Study the drawing (mm; zero at the part's minimum x, y, z) and answer. A direction names the side the tool comes from. Coordinates: 2 decimals unless noted, no trailing zeros. Order: outer loops, then holes, each group sorted by start corner. A loop starts at its lowest first (then second) coordinate and runs counter-clockwise, first axis right, second up. Notation, with made-up numbers: M -27,-24.75 L 27,-24.75 A22 ccw 27,-12.75 Z; hole C -7.75,-37.5 d3. An arc over 180 degrees is marked long. Put each result on its own line as item: value.
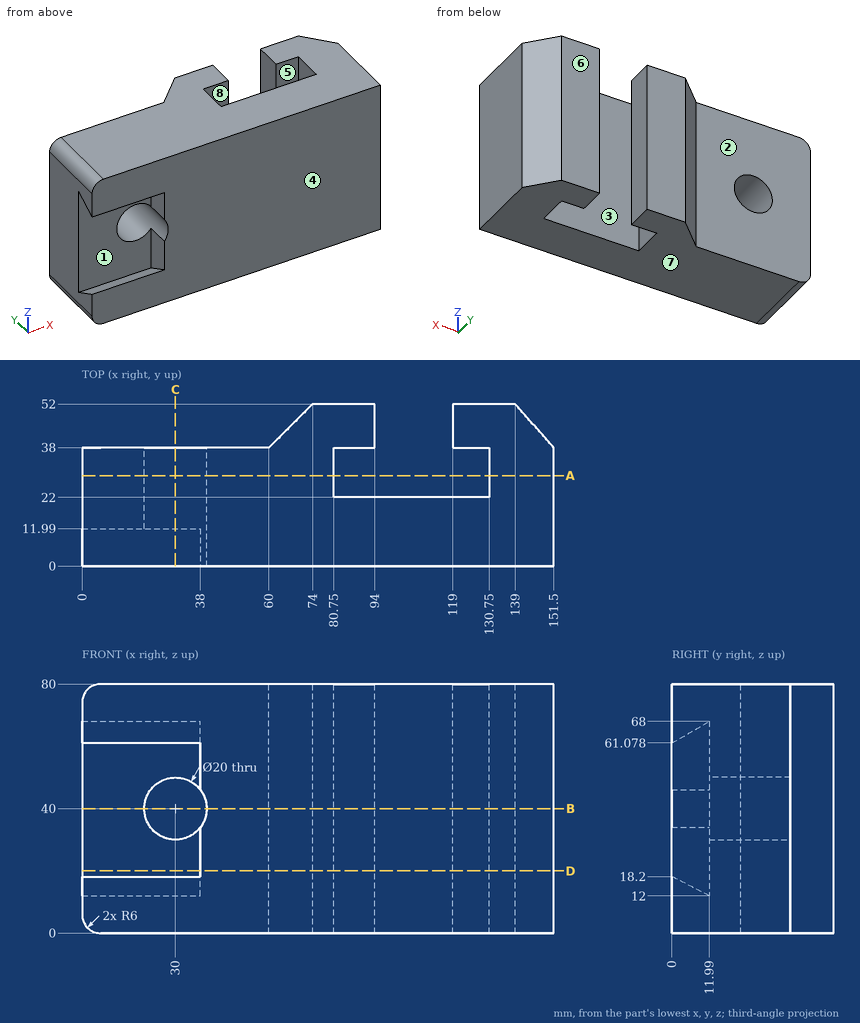
Q1. Consider line 1 along X through (y, z) = (29.5, 40); line 2 along X through (y, z) = (16, 40); line 3 along Y through (x, z) = (88.5, 76). Determine where each line is inside the solid, lowest interval first.
Answers below:
line 1: x = 0 to 20, 40 to 80.75, 130.75 to 151.5
line 2: x = 0 to 20, 40 to 151.5
line 3: y = 0 to 22, 38 to 52
Q2. Find section D-D on z = 20. Write down the section's boundary in (x, y), plus the area to 3 significant figures.
Answers below:
outline: M 0,11.99 L 38,11.99 L 38,0 L 151.5,0 L 151.5,38 L 139,52 L 119,52 L 119,38 L 130.75,38 L 130.75,22 L 80.75,22 L 80.75,38 L 94,38 L 94,52 L 74,52 L 60,38 L 0,38 Z
area: 5,250 mm^2
Q3. Find section B-B on z = 40. Write down the section's boundary in (x, y).
Answers below:
outline: M 0,11.99 L 20,11.99 L 20,38 L 0,38 Z; M 40,0 L 151.5,0 L 151.5,38 L 139,52 L 119,52 L 119,38 L 130.75,38 L 130.75,22 L 80.75,22 L 80.75,38 L 94,38 L 94,52 L 74,52 L 60,38 L 40,38 Z
Q4. Given pin 1 (11 mm diameter, centred on y = 48.5, z = 32.5, fed in from +X) (1 decimal); pin 2 (3.5 mm diameter, centred on y = 4.5, z = 18.5, fed in from -X); pin 3 (12 mm diameter, centred on x = 30, z = 40, fed in from +Y); pin 4 (19 mm diameter, centred on x = 20, z = 39, fed in from -Y), each flat-ended and moving along its own axis, determine where each tip first touches the part or whether it passes through.
Answers below:
pin 1: stops at x = 147
pin 2: stops at x = 38
pin 3: passes through
pin 4: stops at y = 11.99
Q5. Find section A-A on y = 29. Write down the section's boundary in (x, z).
Answers below:
outline: M 0,6 A6 ccw 6,0 L 80.75,0 L 80.75,80 L 6,80 A6 ccw 0,74 Z; M 130.75,0 L 151.5,0 L 151.5,80 L 130.75,80 Z; hole C 30,40 d20
Q6. Find section C-C on x = 30. Write down the section's boundary in (y, z), plus the area to 3 significant figures.
Answers below:
outline: M 0,0 L 38,0 L 38,30 L 11.99,30 L 11.99,12 L 0,18.2 Z; M 0,61.08 L 11.99,68 L 11.99,50 L 38,50 L 38,80 L 0,80 Z
area: 1,930 mm^2
Q7. A tool of negligible diameter and unlimited length cuts with its end or side. For the marked faces 1, 2, 3 and 4, from which of +Z, -Z, +X, -X, +Y, -Y can it reach the whole face along a straight path? Write none if from no direction.
Answers below:
face 1: -X
face 2: +Z, -Z, -X, +Y
face 3: +Z, -Z
face 4: +Z, -Z, +X, -X, -Y
Q8. For a pull along Y with two mould halves and no side action, classify the marked faces 5, 6, 7 and 8 as +Y half, -Y half, draft (parallel to the pull), parting line (faces both ways), or undercut.
Answers below:
face 5: undercut
face 6: +Y half
face 7: draft
face 8: undercut
